Here's how the part is built. I have some questions about the finished solid (model axes, mm). Face numbers are marked on the shaded views. A direction names the side the tool comes from. Round coordinates to 2 decimals unless told otherwise and drop trailing zeros. Loops run counter-clockwise (first coordinate to the right, second up) from the corner with the lowest first, then second, coordinate; pieces in that order, holes last. Notation, with made-up numbers: M 52,61.5 L 85,61.5 A22 cw 85,71.5 Z; hole C 16.5,-28 d6. An arc over 180 degrees is marked long. Answer as CSV lines item,"result".
```python
from build123d import *

# Parameters (mm, degrees)
SKETCH1_W           = 800
SKETCH1_H           = 134
BOSS_EXTRUDE1_DEPTH = 100
SKETCH2_W           = 500
SKETCH2_H           = 200
CUT_EXTRUDE1_DEPTH  = 100
SKETCH3_W           = 110
SKETCH3_H           = 80
CUT_EXTRUDE2_DEPTH  = 80


with BuildPart() as part:
    # Sketch1 → Boss-Extrude1 (new body)
    with BuildSketch(Plane(origin=(0, 0, 0), x_dir=(1, 0, 0), z_dir=(0, 1, 0))):
        Rectangle(SKETCH1_W, SKETCH1_H)
    extrude(amount=BOSS_EXTRUDE1_DEPTH)

    # Sketch2 → Cut-Extrude1 (cut)
    with BuildSketch(Plane(origin=(0, 100, 0), x_dir=(1, 0, 0), z_dir=(0, 1, 0))):
        with Locations((0, -67)):
            Rectangle(SKETCH2_W, SKETCH2_H)
    extrude(amount=-CUT_EXTRUDE1_DEPTH, mode=Mode.SUBTRACT)

    # Sketch3 → Cut-Extrude2 (cut)
    with BuildSketch(Plane(origin=(0, 100, 0), x_dir=(1, 0, 0), z_dir=(0, 1, 0))):
        with Locations((-325, -7)):
            Rectangle(SKETCH3_W, SKETCH3_H)
    cut_extrude2 = extrude(amount=-CUT_EXTRUDE2_DEPTH, mode=Mode.SUBTRACT)

    # Mirror1: Cut-Extrude2 across plane
    add(cut_extrude2.mirror(Plane(origin=(0, 0, 0), x_dir=(0, 0, 1), z_dir=(1, 0, 0))), mode=Mode.SUBTRACT)


solid = part.part
```
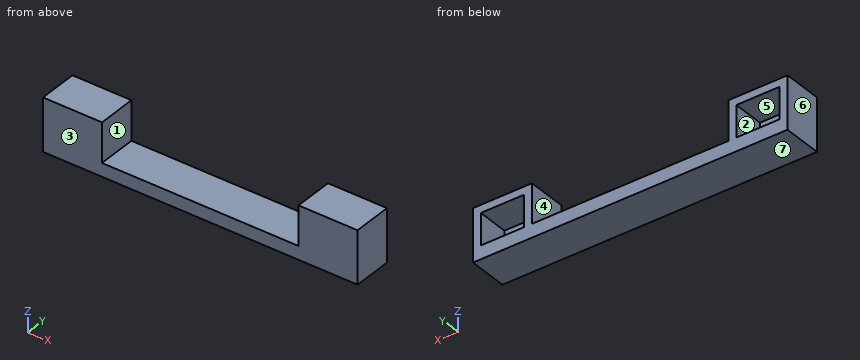
1. If I drill on line 1 (X direction, y = 35.5, z = 14); line 2 (X direction, y = 78, z = 48.5); line 3 (Z direction, x = 163, y = 63.5), over which ranges is the centre line in solid material (lowest first)? Write a range as [from, to].
Evaluation:
line 1,"x = [-400, -380], [-270, -250], [250, 270], [380, 400]"
line 2,"x = [-400, -250], [250, 400]"
line 3,"z = [-67, -33]"
2. I want a section at C-C, the plane x = 341. Please give me the cut outline in (y, z).
Evaluation:
outline,"M 0,-67 L 100,-67 L 100,-33 L 20,-33 L 20,47 L 100,47 L 100,67 L 0,67 Z"
3. We'd pull the mould along X, two halves only. Please class the marked faces 4, 5, 6 and 7: pulls with the +X half, pulls with the -X half, needs draft (parallel to the pull), parting line crosses it, or undercut.
Evaluation:
face 4,"undercut"
face 5,"undercut"
face 6,"pulls with the -X half"
face 7,"needs draft"
4. I want a section at B-B, the plane y = 46. Please give me the cut outline in (x, z), and give its area (3 significant figures).
Evaluation:
outline,"M -400,-67 L 400,-67 L 400,67 L 250,67 L 250,-33 L -250,-33 L -250,67 L -400,67 Z; hole M -380,-33 L -270,-33 L -270,47 L -380,47 Z; hole M 270,-33 L 380,-33 L 380,47 L 270,47 Z"
area,"39,600 mm²"
5. For P1, Ø24, axis at x = -319.5, z = -12, coming from the +Y side, with a flat end and sliding along its axis, tell me the tip position at first contact or that it passes through.
Evaluation:
P1,"stops at y = 20"
6. I want a section at D-D, the plane x = -62. Please give me the cut outline in (y, z).
Evaluation:
outline,"M 0,-67 L 100,-67 L 100,-33 L 0,-33 Z"
7. I want a section at A-A, the plane z = 39. Please give me the cut outline in (x, y).
Evaluation:
outline,"M -400,0 L -250,0 L -250,100 L -270,100 L -270,20 L -380,20 L -380,100 L -400,100 Z; M 250,0 L 400,0 L 400,100 L 380,100 L 380,20 L 270,20 L 270,100 L 250,100 Z"
8. Which directions (+Z, -Z, +X, -X, +Y, -Y) give clear straight access to the entire face, cutting with the end or side of a thin tool? Please do the marked faces 1, 2 and 3.
Evaluation:
face 1,"+Z, +Y, -Y"
face 2,"+Y"
face 3,"+Z, -Z, +X, -X, -Y"
